Verification items for the finished model (mm, model axes). A direction names the side the tool comes from. Give positions to 0.01 mm unless a question says otherwise; leave off trailing zeros. Order: outer loops, then holes, each group sorted by start corner. A loop starts at its lowest first (then second) coordinate and runs counter-clockwise, first axis right, second up. Notation, with made-up numbers: M -5.75,18.25 L 13.25,18.25 A27 ccw 13.25,56.25 Z; hole C 59.25,-24 d4. An arc over 180 degrees is marked long. Answer as a JSON object with one key per item and string values.
```python
from build123d import *

# Parameters (mm, degrees)
SKETCH_1_W             = 115
SKETCH_1_H             = 64
EXTRUDE_1_DEPTH        = 6
SKETCH_2_W             = 60
SKETCH_2_H             = 14
CUT_EXTRUDE_1_DEPTH    = 1.5
SKETCH_3_R             = 2
CUT_EXTRUDE_2_DEPTH    = 67.889834803
CUT_EXTRUDE_3_REACH    = 68.89
HOLE_WIZARD_M6_1_D     = 5
HOLE_WIZARD_M6_1_DEPTH = 18
HOLE_WIZARD_M6_1_TIP   = 1.502151548


with BuildPart() as part:
    # 草图1 → 凸台-拉伸1 (new, symmetric)
    with BuildSketch(Plane.XY):
        Rectangle(SKETCH_1_W, SKETCH_1_H)
    extrude(amount=EXTRUDE_1_DEPTH, both=True)

    # 草图2 → 切除-拉伸1 (cut)
    with BuildSketch(Plane.XY.offset(6)):
        with Locations((0, 25)):
            Rectangle(SKETCH_2_W, SKETCH_2_H)
    cut_extrude_1 = extrude(amount=-CUT_EXTRUDE_1_DEPTH, mode=Mode.SUBTRACT)

    # 草图3 → 切除-拉伸2 (cut, symmetric)
    with BuildSketch(Plane.XY.offset(6)):
        with Locations((-30, 18)):
            Circle(SKETCH_3_R)
        with Locations((30, 18)):
            Circle(SKETCH_3_R)
    cut_extrude_2 = extrude(amount=CUT_EXTRUDE_2_DEPTH, both=True, mode=Mode.SUBTRACT)

    # 镜向1: 切除-拉伸1, 切除-拉伸2 across plane
    add(cut_extrude_1.mirror(Plane.ZX), mode=Mode.SUBTRACT)
    add(cut_extrude_2.mirror(Plane.ZX), mode=Mode.SUBTRACT)

    # 草图4 → 切除-拉伸3 (cut, up to next)
    with BuildSketch(Plane.XY.offset(6), mode=Mode.PRIVATE) as cut_extrude_3_sk1:
        with BuildLine():
            Line((-50.5, 27), (-38.5, 27))
            ThreePointArc((-38.5, 27), (-35.5, 24), (-38.5, 21))
            Line((-38.5, 21), (-50.5, 21))
            ThreePointArc((-50.5, 21), (-53.5, 24), (-50.5, 27))
        make_face()
    cut_extrude_3_tool1 = extrude(cut_extrude_3_sk1.sketch, amount=-CUT_EXTRUDE_3_REACH, mode=Mode.PRIVATE) & part.part
    # 草图4 → 切除-拉伸3 (cut, up to next)
    with BuildSketch(Plane.XY.offset(6), mode=Mode.PRIVATE) as cut_extrude_3_sk2:
        with BuildLine():
            Line((50.5, 27), (38.5, 27))
            ThreePointArc((38.5, 27), (35.5, 24), (38.5, 21))
            Line((38.5, 21), (50.5, 21))
            ThreePointArc((50.5, 21), (53.5, 24), (50.5, 27))
        make_face()
    cut_extrude_3_tool2 = extrude(cut_extrude_3_sk2.sketch, amount=-CUT_EXTRUDE_3_REACH, mode=Mode.PRIVATE) & part.part
    # 草图4 → 切除-拉伸3 (cut, up to next)
    with BuildSketch(Plane.XY.offset(6), mode=Mode.PRIVATE) as cut_extrude_3_sk3:
        with BuildLine():
            Line((-50.5, -27), (-38.5, -27))
            ThreePointArc((-38.5, -27), (-35.5, -24), (-38.5, -21))
            Line((-38.5, -21), (-50.5, -21))
            ThreePointArc((-50.5, -21), (-53.5, -24), (-50.5, -27))
        make_face()
    cut_extrude_3_tool3 = extrude(cut_extrude_3_sk3.sketch, amount=-CUT_EXTRUDE_3_REACH, mode=Mode.PRIVATE) & part.part
    # 草图4 → 切除-拉伸3 (cut, up to next)
    with BuildSketch(Plane.XY.offset(6), mode=Mode.PRIVATE) as cut_extrude_3_sk4:
        with BuildLine():
            Line((50.5, -27), (38.5, -27))
            ThreePointArc((38.5, -27), (35.5, -24), (38.5, -21))
            Line((38.5, -21), (50.5, -21))
            ThreePointArc((50.5, -21), (53.5, -24), (50.5, -27))
        make_face()
    cut_extrude_3_tool4 = extrude(cut_extrude_3_sk4.sketch, amount=-CUT_EXTRUDE_3_REACH, mode=Mode.PRIVATE) & part.part
    add(cut_extrude_3_tool1.solids().sort_by_distance((-44.5, 24, 6))[0], mode=Mode.SUBTRACT)
    add(cut_extrude_3_tool2.solids().sort_by_distance((44.5, 24, 6))[0], mode=Mode.SUBTRACT)
    add(cut_extrude_3_tool3.solids().sort_by_distance((-44.5, -24, 6))[0], mode=Mode.SUBTRACT)
    add(cut_extrude_3_tool4.solids().sort_by_distance((44.5, -24, 6))[0], mode=Mode.SUBTRACT)

    # M6 螺纹孔1
    with Locations(Plane(origin=(57.5, 0, 0), x_dir=(0, 0, 1), z_dir=(1, 0, 0))):
        with Locations((0, 0)):
            Hole(HOLE_WIZARD_M6_1_D / 2, depth=HOLE_WIZARD_M6_1_DEPTH)
            with Locations((0, 0, -(HOLE_WIZARD_M6_1_DEPTH + HOLE_WIZARD_M6_1_TIP / 2))):  # 118° drill point
                Cone(0, HOLE_WIZARD_M6_1_D / 2, HOLE_WIZARD_M6_1_TIP, mode=Mode.SUBTRACT)


solid = part.part
```
Q1. Section check B-B on x = 11. Record the cut outline in (y, z), then the cut area to 3 significant figures.
Resolved:
{"outline": "M -32,-6 L 32,-6 L 32,4.5 L 18,4.5 L 18,6 L -18,6 L -18,4.5 L -32,4.5 Z", "area": "726 mm²"}
Q2. Section check A-A on z = -4. Count the separate pieces of the cut face and the enclosed holes in it, then the cut area to 3 significant figures.
Resolved:
{"separate pieces": "1", "enclosed holes": "8", "area": "6,910 mm²"}
Q3. Gauge pin test, flat ends, axial feed: pin 1 Ø11 at (x, y) = (-1, -24.5) entering from +Z; pin 2 Ø4 at (y, z) = (0, 0) entering from +X; pin 3 Ø3 at (x, y) = (-30, -18) entering from -Z; pin 4 Ø1.2 at (x, z) = (10, 5.5) entering from -Y. Record the tip position at first contact, or that the pin passes through.
Resolved:
{"pin 1": "stops at z = 4.5", "pin 2": "stops at x = 39.2", "pin 3": "passes through", "pin 4": "stops at y = -18"}
Q4. Release check for a two-part mould opening along Z. For faces 4 (the face through (-1, 0, 6)), 5 (the face through (-45, 27, 0)), 6 (the face through (48.37, 2.44, 0.54)) record: +Z half, -Z half, draft (parallel to the pull), parting line (faces both ways), or undercut.
Resolved:
{"face 4": "+Z half", "face 5": "draft", "face 6": "undercut"}
Q5. Material ranges on L1, parallel to Y at x = -42, z = 0.5; L2, parallel to X at y = 18, z = 0.75; L3, parallel to Y at x = 47.5, z = 0, recorded low to high.
Resolved:
{"L1": "y = -32 to -27, -21 to 21, 27 to 32", "L2": "x = -57.5 to -32, -28 to 28, 32 to 57.5", "L3": "y = -32 to -27, -21 to -2.5, 2.5 to 21, 27 to 32"}
Q6. Tool access check on faces 1 (the face through (0, 25, 4.5)), 2 (the face through (0, -25, 4.5)), 3 (the face through (-44, 21, 0)). Record the directions out of +Z, -Z, +X, -X, +Y, -Y that give a thin tool (end or side, any length) a straight path to the whole face; none if there is none.
Resolved:
{"face 1": "+Z, +Y", "face 2": "+Z, -Y", "face 3": "+Z, -Z"}
